The model under review builds one solid part; all positions refer to its coordinate system, in mm. A direction names the side the tool comes from. Round coordinates to 2 decimals unless told otherwise and drop trailing zeros. Order: outer loops, then holes, each group sorted by start corner. A loop starts at its lowest first (then second) coordinate and runs counter-clockwise, first axis right, second up.
1) Consider section B-B (y = 46). Give the boundary of the cut face in (x, z).
2) To check wall thickness, follow L1, parallel to X at y = 18, z = 0; L2, parallel to X at y = 16, z = -61.5; L3, parallel to X at y = 39.5, z = 0. State the ranges of each line that lie inside material, in increasing order.
3) Machinability: for faces 1 (the face through (-59.824, 17.255, 4.589)), 2 (the face through (59.81, 17.26, 4.77)), 3 (the face through (1.32, 42.6, -29.97)), which of the approach directions +Z, -Z, +X, -X, +Y, -Y give a long, thin tool a straight path to every point of the face, cutting with its end or side? Answer none if there is none.
4) Mouldability with a two-part tool opening along Z and no side actions: class faces 4 (the face through (65.191, 17.255, -37.083)), 5 (the face through (0, 42, 68)), 6 (the face through (33.89, 17.26, 49.51)) as pulls with the +Z half, pulls with the -Z half, needs draft (parallel to the pull), parting line crosses it, or undercut.
5) Clearance check with flat-ended pins moving along their axes: P1, Ø9.5, axis at y = 26, z = -62, coming from the -X side; P2, Ø1.5, axis at x = -35.5, y = 25.5, coming from the +Z side; P3, Ø2.5, axis at y = 14.5, z = -62.5, coming from the +X side. State where each tip first meets the part, or that it passes through.
6) Consider section C-C (z = -28). Give the boundary of the cut face in (x, y), then the cut area to 3 significant figures.
7) Consider section A-A (x = 0). Give the boundary of the cut face in (y, z).
8) Consider section D-D (x = -55.5). Give the boundary of the cut face in (y, z), then the cut area to 3 significant figures.
from build123d import *

# Parameters (mm, degrees)
BASE_BODY_35MM_DEPTH          = 35
THREE_LOBE_PROFILE_35MM_DEPTH = 35
RAISED_HUB_15MM_DEPTH         = 15
COUNTERBORE_SKETCH_60_R       = 30
COUNTERBORE_60X15_DEPTH       = 15
BORE_SKETCH_30_R              = 15
THROUGH_BORE_30_DEPTH         = 35


with BuildPart() as part:
    # Base Profile Sketch → Base Body 35mm (new body)
    with BuildSketch(Plane(origin=(0, 0, 0), x_dir=(1, 0, 0), z_dir=(0, 1, 0))):
        with BuildLine():
            ThreePointArc((-41.666435185, 62.361111111), (-64.951905284, 37.5), (-74.839524023, 4.903635799))
            ThreePointArc((-74.839524023, 4.903635799), (-34.641016151, -20), (-33.173088838, -67.264746911))
            ThreePointArc((-33.173088838, -67.264746911), (0, -75), (33.173088838, -67.264746911))
            ThreePointArc((33.173088838, -67.264746911), (34.641016151, -20), (74.839524023, 4.903635799))
            ThreePointArc((74.839524023, 4.903635799), (64.951905284, 37.5), (41.666435185, 62.361111111))
            ThreePointArc((41.666435185, 62.361111111), (0, 40), (-41.666435185, 62.361111111))
        make_face()
    extrude(amount=BASE_BODY_35MM_DEPTH)

    # Lobe Profile Sketch → Three-Lobe Profile 35mm (add)
    with BuildSketch(Plane.XZ):
        with BuildLine():
            Line((20, -56.568542495), (20, -64.992307237))
            ThreePointArc((20, -64.992307237), (0, -68), (-20, -64.992307237))
            Line((-20, -64.992307237), (-20, -56.568542495))
            ThreePointArc((-20, -56.568542495), (-51.961524227, -30), (-58.989794856, 10.963763172))
            Line((-58.989794856, 10.963763172), (-66.284989118, 15.175645543))
            ThreePointArc((-66.284989118, 15.175645543), (-58.889727457, 34), (-46.284989118, 49.816661694))
            Line((-46.284989118, 49.816661694), (-38.989794856, 45.604779323))
            ThreePointArc((-38.989794856, 45.604779323), (0, 60), (38.989794856, 45.604779323))
            Line((38.989794856, 45.604779323), (46.284989118, 49.816661694))
            ThreePointArc((46.284989118, 49.816661694), (58.889727457, 34), (66.284989118, 15.175645543))
            Line((66.284989118, 15.175645543), (58.989794856, 10.963763172))
            ThreePointArc((58.989794856, 10.963763172), (51.961524227, -30), (20, -56.568542495))
        make_face()
    extrude(amount=-THREE_LOBE_PROFILE_35MM_DEPTH)

    # Hub Profile Sketch → Raised Hub 15mm (add)
    with BuildSketch(Plane(origin=(0, 35, 0), x_dir=(1, 0, 0), z_dir=(0, 1, 0))):
        with BuildLine():
            ThreePointArc((-37.386628626, 56.8), (-58.889727457, 34), (-67.883557248, 3.977770152))
            ThreePointArc((-67.883557248, 3.977770152), (-34.641016151, -20), (-30.496928622, -60.777770152))
            ThreePointArc((-30.496928622, -60.777770152), (0, -68), (30.496928622, -60.777770152))
            ThreePointArc((30.496928622, -60.777770152), (34.641016151, -20), (67.883557248, 3.977770152))
            ThreePointArc((67.883557248, 3.977770152), (58.889727457, 34), (37.386628626, 56.8))
            ThreePointArc((37.386628626, 56.8), (0, 40), (-37.386628626, 56.8))
        make_face()
    extrude(amount=RAISED_HUB_15MM_DEPTH)

    # Counterbore Sketch Ø60 → Counterbore Ø60x15 (cut)
    with BuildSketch(Plane(origin=(0, 50, 0), x_dir=(1, 0, 0), z_dir=(0, 1, 0))):
        with Locations(Location((0, 0, 0), (0, 0, 270))):
            Circle(COUNTERBORE_SKETCH_60_R)
    extrude(amount=-COUNTERBORE_60X15_DEPTH, mode=Mode.SUBTRACT)

    # Bore Sketch Ø30 → Through Bore Ø30 (cut)
    with BuildSketch(Plane(origin=(0, 35, 0), x_dir=(1, 0, 0), z_dir=(0, 1, 0))):
        with Locations(Location((0, 0, 0), (0, 0, 270))):
            Circle(BORE_SKETCH_30_R)
    extrude(amount=-THROUGH_BORE_30_DEPTH, mode=Mode.SUBTRACT)


solid = part.part
Answer below:
1. outline: (-67.88, -3.98) arc R68 ccw to (-37.39, -56.8) arc R50 cw to (37.39, -56.8) arc R68 ccw to (67.88, -3.98) arc R50 cw to (30.5, 60.78) arc R68 ccw to (-30.5, 60.78) arc R50 cw to start; hole circle Ø60 at (0, 0)
2. L1: x = -60 to -15, 15 to 60
2. L2: x = -42.93 to -41.08, -20 to 20, 41.08 to 42.93
2. L3: x = -56.15 to -30, 30 to 56.15
3. face 1: -X, +Y, -Y
3. face 2: +X, +Y, -Y
3. face 3: +Y
4. face 4: pulls with the -Z half
4. face 5: pulls with the +Z half
4. face 6: undercut
5. P1: stops at x = -48.45
5. P2: stops at z = 48.91
5. P3: stops at x = 43.28
6. outline: (-69.58, 0) - (69.58, 0) - (69.58, 35) - (61.97, 35) - (61.97, 50) - (10.77, 50) - (10.77, 35) - (-10.77, 35) - (-10.77, 50) - (-61.97, 50) - (-61.97, 35) - (-69.58, 35) - close
6. area: 6,410 mm2
7. outline: (0, -68) - (35, -68) - (35, -40) - (50, -40) - (50, -30) - (35, -30) - (35, -15) - (0, -15) - close; (0, 15) - (35, 15) - (35, 30) - (50, 30) - (50, 68) - (35, 68) - (35, 75) - (0, 75) - close
8. outline: (0, -50.45) - (35, -50.45) - (35, -39.29) - (50, -39.29) - (50, 0.32) - (35, 0.32) - (35, 39.29) - (0, 39.29) - close
8. area: 3,730 mm2
